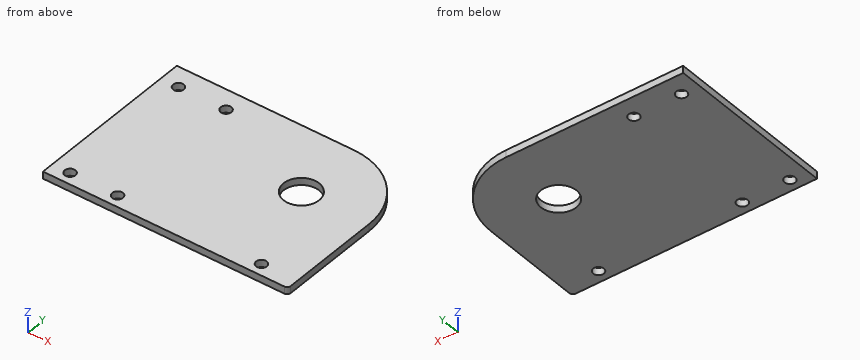
```python
from build123d import *

# Parameters (mm, degrees)
SKETCH_1_W          = 206
SKETCH_1_H          = 145
EXTRUDE_1_DEPTH     = 6
SKETCH_3_R          = 4.5
CUT_EXTRUDE_2_DEPTH = 127.100158604
SKETCH_4_R          = 15
CUT_EXTRUDE_3_DEPTH = 127.100158604
FILLET_1_R          = 57
SKETCH_11_R         = 4.5
CUT_EXTRUDE_6_DEPTH = 127.100158604
FILLET_5_R          = 3


with BuildPart() as part:
    # 草图1 → 凸台-拉伸1 (new body)
    with BuildSketch(Plane.XY):
        Rectangle(SKETCH_1_W, SKETCH_1_H)
    extrude(amount=EXTRUDE_1_DEPTH)

    # 草图3 → 切除-拉伸2 (cut, through all)
    with BuildSketch(Plane.XY.offset(6)):
        with Locations((-88, 55)):
            Circle(SKETCH_3_R)
        with Locations((-48, 55)):
            Circle(SKETCH_3_R)
        with Locations((-88, -62.5)):
            Circle(SKETCH_3_R)
        with Locations((-48, -62.5)):
            Circle(SKETCH_3_R)
    extrude(amount=-CUT_EXTRUDE_2_DEPTH, mode=Mode.SUBTRACT)

    # 草图4 → 切除-拉伸3 (cut, through all)
    with BuildSketch(Plane.XY.offset(6)):
        with Locations((46, 15.5)):
            Circle(SKETCH_4_R)
    extrude(amount=-CUT_EXTRUDE_3_DEPTH, mode=Mode.SUBTRACT)

    # 圆角1
    fillet_1_edges = [part.edges().sort_by_distance(p)[0] for p in [
        (103, 72.5, 3),
    ]]
    fillet(fillet_1_edges, radius=FILLET_1_R)

    # 草图11 → 切除-拉伸6 (cut, through all)
    with BuildSketch(Plane.XY.offset(6)):
        with Locations((73, -62.5)):
            Circle(SKETCH_11_R)
    extrude(amount=-CUT_EXTRUDE_6_DEPTH, mode=Mode.SUBTRACT)

    # 圆角5
    fillet_5_edges = [part.edges().sort_by_distance(p)[0] for p in [
        (103, -72.5, 3),
    ]]
    fillet(fillet_5_edges, radius=FILLET_5_R)


solid = part.part
```
Work out the finished part from the listing and answer in its coordinate system (mm). Give positions to 0.01 mm unless a question says otherwise; leave off trailing zeros. Loops run counter-clockwise (first coordinate to the right, second up) from the corner with the lowest first, then second, coordinate; pieces in that order, holes last. Notation, with made-up numbers: (37, 2) -> (68, 2) arc R6 ccw to (68, 7) -> close; hole circle Ø10 at (-25.75, -38.5). An arc over 180 degrees is marked (long way). Use CSV: the item, a comma, the result in double quotes.
1. The part is cut by section A-A (y = -62.5). Write down the section's boundary in (x, z), then the cut area to 3 significant figures.
Found:
outline,"(-103, 0) -> (-92.5, 0) -> (-92.5, 6) -> (-103, 6) -> close; (-83.5, 0) -> (-52.5, 0) -> (-52.5, 6) -> (-83.5, 6) -> close; (-43.5, 0) -> (68.5, 0) -> (68.5, 6) -> (-43.5, 6) -> close; (77.5, 0) -> (103, 0) -> (103, 6) -> (77.5, 6) -> close"
area,"1,070 mm^2"
2. The part is cut by section C-C (x = 73). Write down the section's boundary in (y, z).
Found:
outline,"(-72.5, 0) -> (-67, 0) -> (-67, 6) -> (-72.5, 6) -> close; (-58, 0) -> (65.7, 0) -> (65.7, 6) -> (-58, 6) -> close"
3. The part is cut by section B-B (x = -48). Write down the section's boundary in (y, z).
Found:
outline,"(-72.5, 0) -> (-67, 0) -> (-67, 6) -> (-72.5, 6) -> close; (-58, 0) -> (50.5, 0) -> (50.5, 6) -> (-58, 6) -> close; (59.5, 0) -> (72.5, 0) -> (72.5, 6) -> (59.5, 6) -> close"
4. The part is cut by section D-D (y = 55). Write down the section's boundary in (x, z).
Found:
outline,"(-103, 0) -> (-92.5, 0) -> (-92.5, 6) -> (-103, 6) -> close; (-83.5, 0) -> (-52.5, 0) -> (-52.5, 6) -> (-83.5, 6) -> close; (-43.5, 0) -> (87.09, 0) -> (87.09, 6) -> (-43.5, 6) -> close"
5. Flat-ended cylindrical pins translate along their axes: pin 1 Ø8 at (x, y) = (61.5, -2.5) entering from -Z; pin 2 Ø7 at (x, y) = (-48, -62.5) entering from -Z; pin 3 Ø2 at (y, z) = (27.5, 3.5) entering from +X. Find the tip coordinate at first contact, or state that the pin passes through.
Found:
pin 1,"z = 0"
pin 2,"through"
pin 3,"x = 101.93"
6. Straight lines are drawn through the part: line 1 (Y direction, x = -88, z = 2.9); line 2 (Y direction, x = 32.5, z = 4.7); line 3 (X direction, y = 50, z = 2.6). For each, find the intervals that lie inside material, in ascending order.
Found:
line 1,"-72.5 to -67, -58 to 50.5, 59.5 to 72.5"
line 2,"-72.5 to 8.96, 22.04 to 72.5"
line 3,"-103 to 91.37"
